Input: dimensioned drawing with shaded views. Units: mm. Origin: part minimum x, y, z. A direction names the side the tool comes from. Round coordinates to 2 decimals unless told otherwise and drop trailing zeros. Write each loop counter-clockwise with the first axis right and the second up, starting at its lowest first coordinate (ties: lowest second). Pieces come first, ordered by that corner, then holes. Notation, with made-up numbers: M 15,50 L 22,50 A19 ccw 22,75 Z; hole C -32,-12.75 d8. An arc over 180 degrees is marked long. Answer in a Markdown table with one row per item. Add a question column.
Item 1: Contact query for flat-ended pins moving along their axis: pin 1 (9 mm diameter, centred on y = 97.5, z = 55, fed in from -X); pin 2 (2 mm diameter, centred on x = 29.5, y = 18, fed in from +Z); pin 3 (1 mm diameter, centred on x = 26, z = 25, fed in from +Y); pin 4 (6 mm diameter, centred on x = 16, y = 49.5, fed in from +Z). Output: stop coordinate, or through.
Item 2: Material intervals for probe 1 along Y at (x, z) = (33.5, 55); probe 2 along Y at (x, z) = (31, 12); probe 3 along X at (y, z) = (65.5, 74), sorted ascending.
Item 3: Set-up query: the marked faces 4, 5 and 6. Return all of +Z, -Z, +X, -X, +Y, -Y with unobstructed straight access to the full face (end or side cutting, diameter ignored); none if empty.
Item 4: Cut plane B-B on z = 12.5. Return loops of the section in (x, y).
Item 5: Mould query, pull axis Z, two halves, no side actions, for the marked faces 1, 2 and 3. Classes: released by +Z, released by -Z, zero draft, split by the parting line, or undercut.
Item 6: Cut plane A-A on y = 55. Return loops of the section in (x, z).
Item 7: Cut plane C-C on x = 27. Return loops of the section in (y, z).
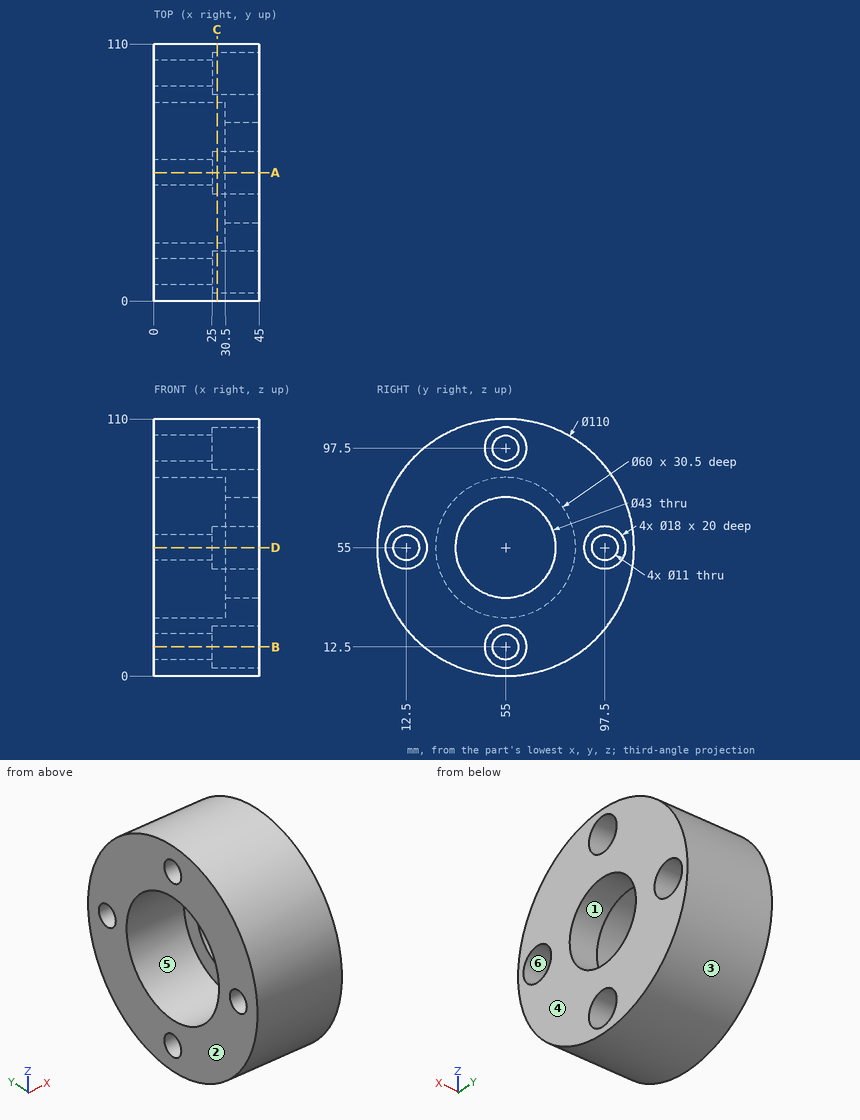
Results below:
| question | item | result |
|---|---|---|
| 1 | pin 1 | through |
| 1 | pin 2 | z = 96.58 |
| 1 | pin 3 | y = 101.42 |
| 1 | pin 4 | z = 109.94 |
| 2 | probe 1 | 0 to 3.5, 21.5 to 33.5, 76.5 to 88.5, 106.5 to 110 |
| 2 | probe 2 | 20.71 to 46.01, 63.99 to 89.29 |
| 2 | probe 3 | 30.5 to 45 |
| 3 | face 4 | +Z, -Z, +X, +Y, -Y |
| 3 | face 5 | -X |
| 3 | face 6 | +X |
| 4 | outline | M 0,20.09 L 45,20.09 L 45,46 L 25,46 L 25,49.5 L 0,49.5 Z; M 0,60.5 L 25,60.5 L 25,64 L 45,64 L 45,89.91 L 0,89.91 Z |
| 5 | face 1 | undercut |
| 5 | face 2 | zero draft |
| 5 | face 3 | split by the parting line |
| 6 | outline | M 0,0 L 45,0 L 45,3.5 L 25,3.5 L 25,7 L 0,7 Z; M 0,18 L 25,18 L 25,21.5 L 45,21.5 L 45,33.5 L 30.5,33.5 L 30.5,25 L 0,25 Z; M 0,85 L 30.5,85 L 30.5,76.5 L 45,76.5 L 45,88.5 L 25,88.5 L 25,92 L 0,92 Z; M 0,103 L 25,103 L 25,106.5 L 45,106.5 L 45,110 L 0,110 Z |
| 7 | outline | C 55,55 d110; hole C 12.5,55 d18; hole C 55,55 d60; hole C 55,12.5 d18; hole C 55,97.5 d18; hole C 97.5,55 d18 |
